Answer from the drawing. Dimensions are ordinates in mm from the lowest x, y and z of the part. Round coordinates to 2 decimals unless told otherwise and drop trailing zeros. Loops run counter-clockwise (first coordinate to the right, second up) from the corner with the lowest first, then second, coordinate; pieces in that order, holes last. Notation, with made-up numbers: (80.25, 2) - (84.25, 2) arc R21 cw to (84.25, 6) - close; hole circle Ø2 at (33.5, -15.75). An arc over 180 degrees is marked (long way). Write item = value, one per line. Start each with the question number.
1) Given pin 1 Ø8 at (x, y) = (18, 14) entering from +Z; pin 2 Ø10 at (x, y) = (17.5, 16.5) entering from -Z; pin 3 Ø6 at (y, z) = (6, 4.5) entering from -X; pin 4 Ø7 at (x, z) = (10.5, 10.5) entering from -Y, each flat-ended and moving along its own axis, determine where each tip first touches the part or whether it passes through.
2) For a pull along Z with two mould halves and no side action, classify the marked faces 1, 2 and 3 as released by +Z, released by -Z, zero draft, split by the parting line, or undercut.
3) Straight lines are drawn through the part: line 1 along X through (y, z) = (20, 10.5); line 2 along Z through (x, y) = (9.5, 10); line 3 along X through (y, z) = (19, 8). For each, find the intervals that lie inside material, in ascending order.
4) Section A-A, the plane x = 10.5 is taken. Determine the outline of the cut face in (y, z), and give its area (3 significant figures).
5) Section B-B, the plane y = 15.75 is taken. Determine the outline of the cut face in (x, z).
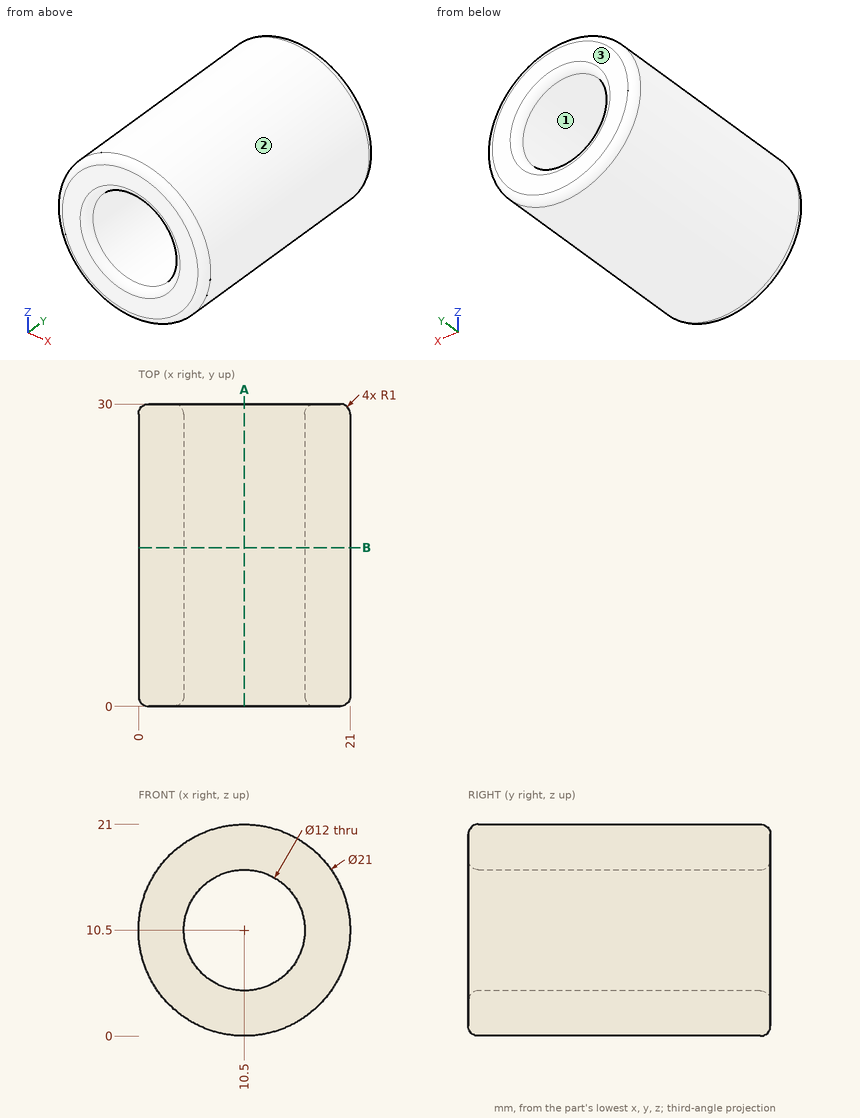
Geometry check:
q1.pin_1 = 20.4
q1.pin_2 = 0.19
q1.pin_3 = 0.44
q1.pin_4 = through
q2.face_1 = undercut
q2.face_2 = split by the parting line
q2.face_3 = zero draft
q3.line_1 = 0 to 4.5, 16.5 to 21
q3.line_2 = 0.05 to 4.58, 16.42 to 20.95
q3.line_3 = 0.3 to 5.05, 15.95 to 20.7
q4.outline = (0, 1) arc R1 ccw to (1, 0) - (29, 0) arc R1 ccw to (30, 1) - (30, 3.5) arc R1 ccw to (29, 4.5) - (1, 4.5) arc R1 ccw to (0, 3.5) - close; (0, 17.5) arc R1 ccw to (1, 16.5) - (29, 16.5) arc R1 ccw to (30, 17.5) - (30, 20) arc R1 ccw to (29, 21) - (1, 21) arc R1 ccw to (0, 20) - close
q4.area = 268 mm2
q5.outline = circle Ø21 at (10.5, 10.5); hole circle Ø12 at (10.5, 10.5)
